from build123d import *

# Parameters (mm, degrees)
SKETCH_1_W              = 42
SKETCH_1_H              = 10
EXTRUDE_1_DEPTH         = 8
SKETCH_2_W              = 22
SKETCH_2_H              = 10
EXTRUDE_2_DEPTH         = 21
SKETCH_3_R              = 6
CUT_EXTRUDE_1_DEPTH     = 38.175260591
HOLE_WIZARD_4_5_4_5_2_D = 4.5
HOLE_WIZARD_M4_1_D      = 3.3
FILLET_3_R              = 3
CHAMFER_1_SIZE          = 1


with BuildPart() as part:
    # 草图1 → 凸台-拉伸1 (new body)
    with BuildSketch(Plane.XY):
        Rectangle(SKETCH_1_W, SKETCH_1_H)
    extrude(amount=EXTRUDE_1_DEPTH)

    # 草图2 → 凸台-拉伸2 (add)
    with BuildSketch(Plane.XY.offset(8)):
        Rectangle(SKETCH_2_W, SKETCH_2_H)
    extrude(amount=EXTRUDE_2_DEPTH)

    # 草图3 → 切除-拉伸1 (cut, through all)
    with BuildSketch(Plane(origin=(0, 5, 0), x_dir=(1, 0, 0), z_dir=(0, 1, 0))):
        with Locations(Location((0, -21, 0), (0, 0, 270))):
            Circle(SKETCH_3_R)
    extrude(amount=-CUT_EXTRUDE_1_DEPTH, mode=Mode.SUBTRACT)

    # Ø4.5 (4.5) 直径孔2 (through all)
    with Locations(Plane.XY.offset(8)):
        with Locations((-16, 0), (16, 0)):
            Hole(HOLE_WIZARD_4_5_4_5_2_D / 2)

    # M4 螺纹孔1 (through all)
    with Locations(Plane(origin=(11, 0, 0), x_dir=(0, 0, -1), z_dir=(1, 0, 0))):
        with Locations((-21, 0)):
            Hole(HOLE_WIZARD_M4_1_D / 2)

    # 圆角3
    fillet_3_edges = [part.edges().sort_by_distance(p)[0] for p in [
        (-11, 0, 29),
        (11, 0, 29),
    ]]
    fillet(fillet_3_edges, radius=FILLET_3_R)

    # 倒角1
    chamfer_1_edges = [part.edges().sort_by_distance(p)[0] for p in [
        (21, -5, 4),
        (21, 5, 4),
        (-21, -5, 4),
        (-21, 5, 4),
    ]]
    chamfer(chamfer_1_edges, length=CHAMFER_1_SIZE)


solid = part.part
Could you check a few things on this model? Use its own coordinates, in mm. A direction names the side the tool comes from. Coordinates: 2 decimals unless noted, no trailing zeros. Loops run counter-clockwise (first coordinate to the right, second up) from the corner with the lowest first, then second, coordinate; pieces in that order, holes last.
1. For P1, Ø2, axis at x = 3, z = 16, coming from the -Y side; P2, Ø5, axis at x = 17.5, y = -1.5, coming from the +Z side; P3, Ø3, axis at y = -0.5, z = 18, coming from the +X side; P4, Ø1, axis at y = -1, z = 18.5, coming from the -X side, each with a flat end and sliding along its axis, tell me the tip position at first contact or that it passes through.
2. Imagine slicing it at C-C (y = -3). Please give me the cut outline in (x, z), and give its area (3 significant figures).
3. I need wall thicknesses on L1, parallel to Y at x = -16, z = 3; L2, parallel to Y at x = 9.7, z = 21; L3, parallel to X at y = -1.5, z = 5.5. Which ranges of each line are inside material? Lowest first, please.
4. Imagine slicing it at A-A (z = 21). Please give me the cut outline in (x, y), and give its area (3 significant figures).
5. Imagine slicing it at D-D (z = 4.75). Please give me the cut outline in (x, y), and give its area (3 significant figures).
6. For faces 1 (the face through (11, 0, 17)), 2 (the face through (-15, -2.2, 8)), 3 (the face through (-18.146, 0.676, 3.944)), which set-ups out of +Z, -Z, +X, -X, +Y, -Y let a thin tool reach every point of the face, with its end or its side?
7. Imagine slicing it at B-B (x = 0). Please give me the cut outline in (y, z).
8. We'd pull the mould along X, two halves only. Please class faces 4 (the face through (13.854, 0.676, 3.944)), 5 (the face through (-20.5, -4.5, 3.9)), 6 (the face through (0, 0, 0)): released by +X, released by -X, zero draft, split by the parting line, or undercut.
Computed values:
1. P1: stops at y = -5
1. P2: stops at z = 8
1. P3: stops at x = 11
1. P4: stops at x = -11
2. outline: (-21, 0) - (21, 0) - (21, 8) - (11, 8) - (11, 26) arc R3 ccw to (8, 29) - (-8, 29) arc R3 ccw to (-11, 26) - (-11, 8) - (-21, 8) - close; hole circle Ø12 at (0, 21)
2. area: 681 mm2
3. L1: y = -5 to -2.25, 2.25 to 5
3. L2: y = -5 to -1.65, 1.65 to 5
3. L3: x = -21 to -17.68, -14.32 to 14.32, 17.68 to 21
4. outline: (-11, -5) - (-6, -5) - (-6, -1.65) - (-11, -1.65) - close; (-11, 1.65) - (-6, 1.65) - (-6, 5) - (-11, 5) - close; (6, -5) - (11, -5) - (11, -1.65) - (6, -1.65) - close; (6, 1.65) - (11, 1.65) - (11, 5) - (6, 5) - close
4. area: 67.0 mm2
5. outline: (-21, -4) - (-20, -5) - (20, -5) - (21, -4) - (21, 4) - (20, 5) - (-20, 5) - (-21, 4) - close; hole circle Ø4.5 at (-16, 0); hole circle Ø4.5 at (16, 0)
5. area: 386 mm2
6. face 1: +Z, +X, +Y, -Y
6. face 2: +Z, -X, +Y, -Y
6. face 3: +Z, -Z
7. outline: (-5, 0) - (5, 0) - (5, 15) - (-5, 15) - close; (-5, 27) - (5, 27) - (5, 29) - (-5, 29) - close
8. face 4: undercut
8. face 5: released by -X
8. face 6: zero draft
